The listing builds one solid part. Answer for the finished solid, in the listing's coordinates (mm). Face numbers are marked on the shaded views. A direction names the side the tool comes from. Round coordinates to 2 decimals unless told otherwise and drop trailing zeros. Write each loop counter-clockwise with the first axis right and the second up, starting at its lowest first coordinate (ties: lowest second). Pieces come first, ordered by that corner, then holes. Notation, with made-up numbers: (-0.75, -0.5) - (11.25, -0.5) arc R29 cw to (11.25, 38.5) - close; hole circle Ø11 at (6.25, 47). An arc over 180 degrees is marked (long way). Answer in a Markdown table with one row per item.
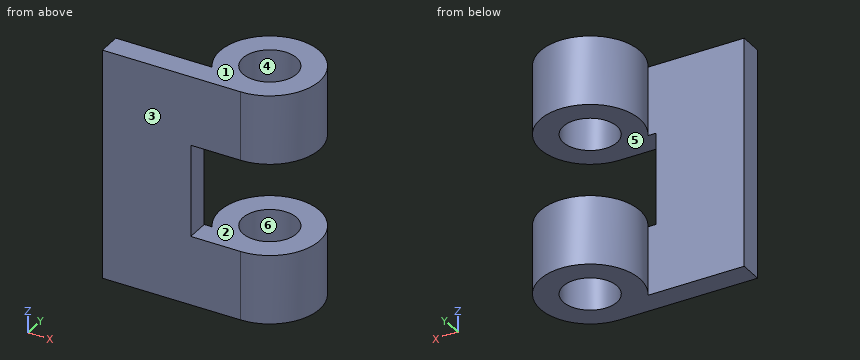
from build123d import *

# Parameters (mm, degrees)
SKETCH_1_R          = 3.5
EXTRUDE_1_DEPTH     = 30
SKETCH_2_W          = 19.333042973
SKETCH_2_H          = 12
CUT_EXTRUDE_1_DEPTH = 15


with BuildPart() as part:
    # 草图1 → 凸台-拉伸1 (new body)
    with BuildSketch(Plane.XY):
        with BuildLine():
            Line((-9, 1.5), (3.522774425, 1.5))
            ThreePointArc((3.522774425, 1.5), (12.122498999, 10.700877125), (9, -1.5))
            Line((9, -1.5), (-9, -1.5))
            Line((-9, -1.5), (-9, 1.5))
        make_face()
        with Locations((9, 5)):
            Circle(SKETCH_1_R, mode=Mode.SUBTRACT)
    extrude(amount=EXTRUDE_1_DEPTH)

    # 草图2 → 切除-拉伸1 (cut, symmetric)
    with BuildSketch(Plane(origin=(0, 0, 0), x_dir=(1, 0, 0), z_dir=(0, 1, 0))):
        with Locations((12.166521487, -15)):
            Rectangle(SKETCH_2_W, SKETCH_2_H)
    extrude(amount=CUT_EXTRUDE_1_DEPTH, both=True, mode=Mode.SUBTRACT)


solid = part.part
(1) Section C-C (x = 8) is taken. Give the vertices of the cut face in (y, z), and give its area (3 significant figures).
Checked values:
| item | result |
|---|---|
| outline | (-1.5, 0) - (1.65, 0) - (1.65, 9) - (-1.5, 9) - close; (-1.5, 21) - (1.65, 21) - (1.65, 30) - (-1.5, 30) - close; (8.35, 0) - (11.42, 0) - (11.42, 9) - (8.35, 9) - close; (8.35, 21) - (11.42, 21) - (11.42, 30) - (8.35, 30) - close |
| area | 112 mm2 |
(2) For a pull along Y with two mould halves and no side action, classify the marked faces 3, 4, 5 and 6 as pulls with the +Y half, pulls with the -Y half, needs draft (parallel to the pull), parting line crosses it, or undercut.
Checked values:
| item | result |
|---|---|
| face 3 | pulls with the -Y half |
| face 4 | undercut |
| face 5 | needs draft |
| face 6 | undercut |
(3) Section D-D (y = -0.5) is taken. Give the vertices of the cut face in (x, z).
Checked values:
| item | result |
|---|---|
| outline | (-9, 0) - (12.46, 0) - (12.46, 9) - (2.5, 9) - (2.5, 21) - (12.46, 21) - (12.46, 30) - (-9, 30) - close |
(4) Section B-B (z = 21.5) is taken. Give the vertices of the cut face in (x, y).
Checked values:
| item | result |
|---|---|
| outline | (-9, -1.5) - (9, -1.5) arc R6.5 ccw (long way) to (3.52, 1.5) - (-9, 1.5) - close; hole circle Ø7 at (9, 5) |
(5) Flat-ended cylindrical pins translate along their axes: pin 1 (2 mm diameter, centred on y = 6.5, z = 9.5, fed in from -X); pin 2 (6.5 mm diameter, centred on x = -3, z = 13, fed in from +Y); pin 3 (1.5 mm diameter, centred on y = 0, z = 12.5, fed in from +X). Find the tip coordinate at first contact, or state that the pin passes through.
Checked values:
| item | result |
|---|---|
| pin 1 | stops at x = 2.53 |
| pin 2 | stops at y = 1.5 |
| pin 3 | stops at x = 2.5 |
(6) For the marked faces 1 and 2, determine the directions among +Z, -Z, +X, -X, +Y, -Y from which every point of the face is accessible in a straight line to the end or side of a thin tool.
Checked values:
| item | result |
|---|---|
| face 1 | +Z, +X, -X, +Y, -Y |
| face 2 | +X, +Y, -Y |
(7) Find the intervals of material crossed by line 1 (Z direction, x = 6, y = 3); line 2 (X direction, y = 5, z = 3.5); line 3 (Y direction, x = -2.5, z = 6.25), in increasing order.
Checked values:
| item | result |
|---|---|
| line 1 | z = 0 to 9, 21 to 30 |
| line 2 | x = 2.5 to 5.5, 12.5 to 15.5 |
| line 3 | y = -1.5 to 1.5 |
(8) Section A-A (y = 5) is taken. Give the vertices of the cut face in (x, z).
Checked values:
| item | result |
|---|---|
| outline | (2.5, 0) - (5.5, 0) - (5.5, 9) - (2.5, 9) - close; (2.5, 21) - (5.5, 21) - (5.5, 30) - (2.5, 30) - close; (12.5, 0) - (15.5, 0) - (15.5, 9) - (12.5, 9) - close; (12.5, 21) - (15.5, 21) - (15.5, 30) - (12.5, 30) - close |
